Can you work these out from the model? Positions are in its coordinate system, mm. A direction names the side the tool comes from. Give positions to 0.01 mm unless a question says otherwise; leave off trailing zeros. Write each loop counter-clockwise with the first axis right and the second up, starting at its lowest first coordinate (ties: lowest second). Pieces come first, ordered by that corner, then holes. Notation, with made-up numbers: (49.5, 7.25) -> (88.5, 7.25) arc R36 cw to (88.5, 42.25) -> close; hole circle Ø6 at (69, 49). An arc over 180 degrees is marked (long way). One line per item, written item: value.
from build123d import *

# Parameters (mm, degrees)
SKETCH1_R           = 25
SKETCH1_R_2         = 12.5
BOSS_EXTRUDE1_DEPTH = 17
MOVE_FACE1_BY       = 7.981500203
SKETCH2_W           = 5
SKETCH2_H           = 4.6
CUT_EXTRUDE1_DEPTH  = 37.487440834


with BuildPart() as part:
    # Sketch1 → Boss-Extrude1 (new body)
    with BuildSketch(Plane.XY):
        Circle(SKETCH1_R)
        Circle(SKETCH1_R_2, mode=Mode.SUBTRACT)
    extrude(amount=-BOSS_EXTRUDE1_DEPTH)

    # Move Face1: a face moved inward by 7.9815
    extrude(part.faces().sort_by_distance((0, -20, 0))[0], amount=MOVE_FACE1_BY, dir=(0, 0, -1), mode=Mode.SUBTRACT)

    # Sketch2 → Cut-Extrude1 (cut, through all)
    with BuildSketch(Plane(origin=(0, 0, -17), x_dir=(-1, 0, 0), z_dir=(0, 0, -1))):
        with Locations((0, 12.5)):
            Rectangle(SKETCH2_W, SKETCH2_H)
    extrude(amount=-CUT_EXTRUDE1_DEPTH, mode=Mode.SUBTRACT)


solid = part.part
1) I need wall thicknesses on L1, parallel to X at y = 9, z = -16.5; L2, parallel to X at y = -1.5, z = -16.5; L3, parallel to Y at x = 3, z = -9.75. Which ranges of each line are inside material? Lowest first, please.
Answer list:
L1: x = -23.32 to -8.67, 8.67 to 23.32
L2: x = -24.95 to -12.41, 12.41 to 24.95
L3: y = -24.82 to -12.13, 12.13 to 24.82
2) For faces 1 (the face through (-11.5, 5.9, -17)), 2 (the face through (2.5, 14, -13)), which set-ups out of +Z, -Z, +X, -X, +Y, -Y let a thin tool reach every point of the face, with its end or its side?
Answer list:
face 1: -Z, +X, -X, +Y, -Y
face 2: +Z, -Z
3) We'd pull the mould along Y, two halves only. Please class faces 3 (the face through (-11.5, 5.9, -7.982)), 4 (the face through (-2.5, 14, -13)), 5 (the face through (23.846, 7.509, -12.428)): released by +Y, released by -Y, zero draft, split by the parting line, or undercut.
Answer list:
face 3: zero draft
face 4: undercut
face 5: split by the parting line
4) If we section it at B-B (x = 0): Write out the boundary of the cut face in (y, z), and give its area (3 significant figures).
Answer list:
outline: (-25, -17) -> (-12.5, -17) -> (-12.5, -7.98) -> (-25, -7.98) -> close; (14.8, -17) -> (25, -17) -> (25, -7.98) -> (14.8, -7.98) -> close
area: 205 mm^2
5) If we section it at A-A (y = 0): Write out the boundary of the cut face in (x, z).
Answer list:
outline: (-25, -17) -> (-12.5, -17) -> (-12.5, -7.98) -> (-25, -7.98) -> close; (12.5, -17) -> (25, -17) -> (25, -7.98) -> (12.5, -7.98) -> close
6) Will these pins go through, and if not, where does the flat tip stop? pin 1 (3 mm diameter, centred on y = 13.5, z = -14.5, fed in from -X); pin 2 (3 mm diameter, centred on y = -19, z = -11.5, fed in from -X); pin 3 (2 mm diameter, centred on y = 13.5, z = -14.5, fed in from +X); pin 4 (15 mm diameter, centred on x = 0, y = 0, fed in from +Z).
Answer list:
pin 1: stops at x = -21.93
pin 2: stops at x = -17.85
pin 3: stops at x = 21.65
pin 4: passes through
7) If we section it at D-D (y = -15): Write out the boundary of the cut face in (x, z).
Answer list:
outline: (-20, -17) -> (20, -17) -> (20, -7.98) -> (-20, -7.98) -> close
8) If we section it at C-C (z = -15.5): Write out the boundary of the cut face in (x, y).
Answer list:
outline: circle Ø50 at (0, 0); hole (-2.5, 12.25) arc R12.5 ccw (long way) to (2.5, 12.25) -> (2.5, 14.8) -> (-2.5, 14.8) -> close
